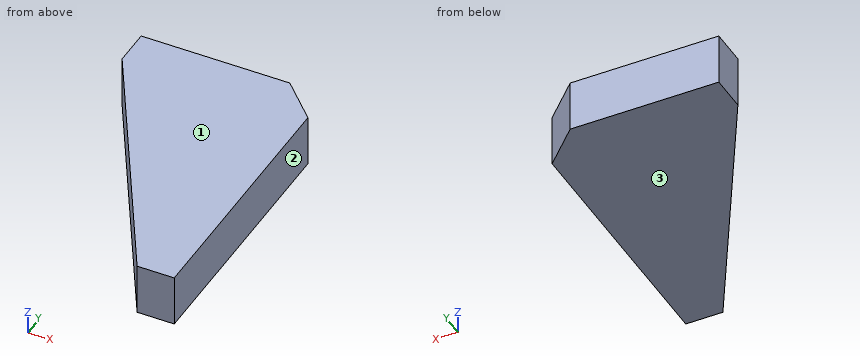
from build123d import *

# Parameters (mm, degrees)
BOSS_EXTRUDE1_DEPTH = 14
CHAMFER1_SIZE       = 10


with BuildPart() as part:
    # Sketch1 → Boss-Extrude1 (new body)
    with BuildSketch(Plane(origin=(0, 0, 0), x_dir=(1, 0, 0), z_dir=(0, 0, -1))):
        Polygon((0, 0), (0, 80), (-10, 80), (-50, 10), (-50, 0), align=None)
    extrude(amount=BOSS_EXTRUDE1_DEPTH)

    # Chamfer1
    chamfer1_edges = [part.edges().sort_by_distance(p)[0] for p in [
        (0, 0, -7),
    ]]
    chamfer(chamfer1_edges, length=CHAMFER1_SIZE)


solid = part.part
Could you check a few things on this model? Use its own coordinates, in mm. Face numbers are marked on the shaded views. Round coordinates to 2 decimals unless told otherwise and drop trailing zeros. Write each loop counter-clockwise with the first axis right and the second up, starting at its lowest first coordinate (ties: lowest second). Pieces come first, ordered by that corner, then holes. Notation, with made-up numbers: (80, 62.25) - (84, 62.25) arc R33 cw to (84, 97.25) - close; hole circle Ø6 at (22.25, 11). An arc over 180 degrees is marked (long way). Put each result on its own line as item: value. Start each with the question number.
(1) I want a section at C-C, the plane x = -17. Please give me the cut outline in (y, z).
(2) Will this pin go through, and if not, where does the flat tip stop? pin 1 (2 mm diameter, centred on x = -30, z = -9.5, fed in from -Y).
(3) I need wall thicknesses on probe 1 along X at (y, z) = (-52, -7.25); probe 2 along Y at (x, z) = (-31.5, -8) (3 decimals); probe 3 along X at (y, z) = (-62.5, -2.5). Which ranges of each line are inside material? Lowest first, please.
(4) Thinking about a two-plate mould opening in Z: for the marked faces 1, 2 and 3, which applies, released by +Z, released by -Z, zero draft, split by the parting line, or undercut?
(5) I want a section at B-B, the plane y = -24. Please give me the cut outline in (x, z), plus the area to 3 significant figures.
(6) I want a section at A-A, the plane z = -1.5. Please give me the cut outline in (x, y).
Here are the results:
1. outline: (-67.75, -14) - (0, -14) - (0, 0) - (-67.75, 0) - close
2. pin 1: stops at y = -46.75
3. probe 1: x = -26 to 0
3. probe 2: y = -42.375 to 0
3. probe 3: x = -20 to 0
4. face 1: released by +Z
4. face 2: zero draft
4. face 3: released by -Z
5. outline: (-42, -14) - (0, -14) - (0, 0) - (-42, 0) - close
5. area: 588 mm^2
6. outline: (-50, -10) - (-10, -80) - (0, -80) - (0, -10) - (-10, 0) - (-50, 0) - close
